Here's how the part is built. I have some questions about the finished solid (model axes, mm). A direction names the side the tool comes from. Round coordinates to 2 decimals unless told otherwise and drop trailing zeros. Write each loop counter-clockwise with the first axis right and the second up, starting at its lowest first coordinate (ties: lowest second). Pieces come first, ordered by that corner, then holes. Notation, with made-up numbers: (85.5, -35.75) -> (114.5, -35.75) arc R30 ccw to (114.5, -9.75) -> close; hole circle Ø11 at (51.5, 45.5). An arc over 180 degrees is marked (long way). Answer as CSV lines item,"result".
from build123d import *

# Parameters (mm, degrees)
LINK_PLATE_PROFILE_R = 2.5
LINK_PLATE_PROFILE_W = 10
LINK_PLATE_PROFILE_H = 10
LINK_PLATE_5MM_DEPTH = 2.5


with BuildPart() as part:
    # Link Plate Profile → Link Plate 5mm (new, symmetric)
    # profile 1 of 4: a face of its own
    with BuildSketch(Plane.XY):
        with BuildLine():
            Line((-45, -5), (10, -5))
            Line((10, -5), (10, 5))
            Line((10, 5), (-45, 5))
            ThreePointArc((-45, 5), (-50, 0), (-45, -5))
        make_face()
        with Locations((-45, 0)):
            Circle(LINK_PLATE_PROFILE_R, mode=Mode.SUBTRACT)
    # profile 2 of 4: a face of its own
    with BuildSketch(Plane.XY):
        with Locations((15, 0)):
            Rectangle(LINK_PLATE_PROFILE_W, LINK_PLATE_PROFILE_H)
    # profile 3 of 4: a face of its own
    with BuildSketch(Plane.XY):
        with BuildLine():
            Line((20, -5), (45, -5))
            ThreePointArc((45, -5), (50, 0), (45, 5))
            Line((45, 5), (20, 5))
            Line((20, 5), (20, -5))
        make_face()
        with Locations((45, 0)):
            Circle(LINK_PLATE_PROFILE_R, mode=Mode.SUBTRACT)
    # profile 4 of 4: a face of its own
    with BuildSketch(Plane.XY):
        with BuildLine():
            Line((20, -16), (20, -5))
            Line((20, -5), (10, -5))
            Line((10, -5), (10, -16))
            ThreePointArc((10, -16), (15, -21), (20, -16))
        make_face()
        with Locations((15, -16)):
            Circle(LINK_PLATE_PROFILE_R, mode=Mode.SUBTRACT)
    extrude(amount=LINK_PLATE_5MM_DEPTH, both=True)


solid = part.part
Item 1: Suppose I cut it at A-A, the plane x = 15. List the corners of the cut face in (y, z) for me, then the cut area to 3 significant figures.
Results found:
outline,"(-21, -2.5) -> (-18.5, -2.5) -> (-18.5, 2.5) -> (-21, 2.5) -> close; (-13.5, -2.5) -> (5, -2.5) -> (5, 2.5) -> (-13.5, 2.5) -> close"
area,"105 mm²"
Item 2: I need wall thicknesses on L1, parallel to Y at x = 15, z = -1.4; L2, parallel to Y at x = -45, z = -0.85; L3, parallel to X at y = 1.5, z = -0.25. Which ranges of each line are inside material? Lowest first, please.
Results found:
L1,"y = -21 to -18.5, -13.5 to 5"
L2,"y = -5 to -2.5, 2.5 to 5"
L3,"x = -49.77 to -47, -43 to 43, 47 to 49.77"
Item 3: Suppose I cut it at C-C, the plane y = 0. List the corners of the cut face in (x, z) for me.
Results found:
outline,"(-50, -2.5) -> (-47.5, -2.5) -> (-47.5, 2.5) -> (-50, 2.5) -> close; (-42.5, -2.5) -> (42.5, -2.5) -> (42.5, 2.5) -> (-42.5, 2.5) -> close; (47.5, -2.5) -> (50, -2.5) -> (50, 2.5) -> (47.5, 2.5) -> close"
Item 4: Suppose I cut it at D-D, the plane x = -34.5. List the corners of the cut face in (y, z) for me, then the cut area to 3 significant figures.
Results found:
outline,"(-5, -2.5) -> (5, -2.5) -> (5, 2.5) -> (-5, 2.5) -> close"
area,"50.0 mm²"
Item 5: Suppose I cut it at B-B, the plane z = -1.35. List the corners of the cut face in (x, y) for me, then the cut area to 3 significant figures.
Results found:
outline,"(-45, -5) -> (10, -5) -> (10, -16) arc R5 ccw to (20, -16) -> (20, -5) -> (45, -5) arc R5 ccw to (45, 5) -> (-45, 5) arc R5 ccw to start; hole circle Ø5 at (-45, 0); hole circle Ø5 at (15, -16); hole circle Ø5 at (45, 0)"
area,"1,070 mm²"
Item 6: If we mould it in two halves opening along X, with no side actions, what happens to faces 4 (the cylindrical face through (47.31, -0.96, -0.04)), 5 (the flat face through (-1, -2, 2.5)), 6 (the flat face through (20, -11, 0)), 7 (the cylindrical face through (12.5, -15.9, 0))? For each: pulls with the +X half, pulls with the -X half, needs draft (parallel to the pull), parting line crosses it, or undercut.
Results found:
face 4,"undercut"
face 5,"needs draft"
face 6,"pulls with the +X half"
face 7,"undercut"
Item 7: Will this pin go through, and if not, where does the flat tip stop? pin 1 (3 mm diameter, centred on y = -14, z = 0, fed in from -X).
Results found:
pin 1,"stops at x = 10"
Item 8: For faces 1 (the flat face through (32, -5, 0)), 2 (the flat face through (-18, -5, 0)), 3 (the cylindrical face through (-50, 0, 0)), which set-ups out of +Z, -Z, +X, -X, +Y, -Y let a thin tool reach every point of the face, with its end or its side?
Results found:
face 1,"+Z, -Z, +X, -Y"
face 2,"+Z, -Z, -X, -Y"
face 3,"+Z, -Z, -X"
